Design review of the part built by this model. Coordinates are the model's own, in mm. Face numbers are marked on the shaded views. A direction names the side the tool comes from. Coordinates: 2 decimals unless noted, no trailing zeros. Write each loop counter-clockwise with the first axis right and the second up, starting at its lowest first coordinate (ties: lowest second). Pieces come first, ordered by that corner, then holes.
Q1. For L1, parallel to Y at x = 0, z = 4; L2, parallel to X at y = 14, z = 2.25; L3, parallel to Y at x = -35, z = 6.5, list the stretches that pass through material, from the lowest coordinate up.
Q2. Take a section at A-A, the plane x = 0. Write out the cut boundary in (y, z), plus the area to 3 significant figures.
Q3. For the marked faces 5, 6 and 7, list the 3-axis set-ups (+Z, -Z, +X, -X, +Y, -Y) from which the entire face can be reached by the end or side of a thin tool; tool diameter is ignored.
Q4. Take a section at B-B, the plane z = 4.5. Write out the cut boundary in (x, y), plus the area to 3 significant figures.
Q5. The part is to be moulded in two halves that separate along X. For the marked faces 1, 2, 3 and 4, say which applies: released by +X, released by -X, zero draft, split by the parting line, or undercut.
Q6. For pin 1 Ø5 at (y, z) = (-25.5, 8.5) entering from +X; pin 2 Ø3 at (x, z) = (-21.5, 4.5) entering from +Y; pin 3 Ø3 at (y, z) = (-28.5, 3) entering from -X, all flat-tipped, find the tip position at first contact; note any pin that passes through.
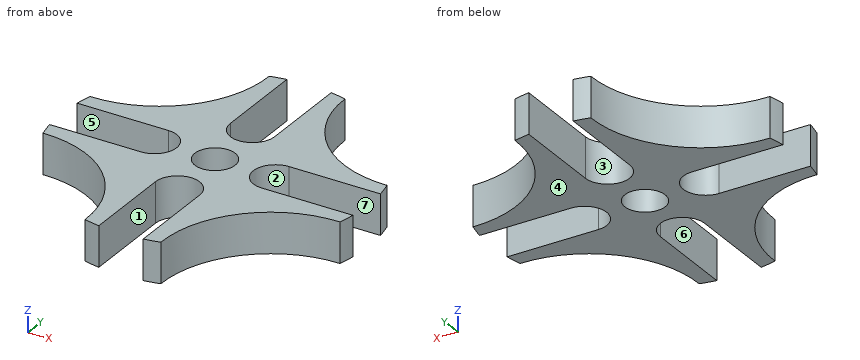
from build123d import *

# Parameters (mm, degrees)
SPIDER_PLATE_PROFILE_R          = 5
SPIDER_PLATE_EXTRUDE_10MM_DEPTH = 10


with BuildPart() as part:
    # Spider Plate Profile → Spider Plate Extrude 10mm (new body)
    with BuildSketch(Plane.XY):
        with BuildLine():
            Line((5.5, -15), (5.5, -37.599867021))
            ThreePointArc((5.5, -37.599867021), (7.46440512, -37.259665272), (9.408264389, -36.816905916))
            ThreePointArc((9.408264389, -36.816905916), (17.313241035, -17.313241035), (36.816905916, -9.408264389))
            ThreePointArc((36.816905916, -9.408264389), (37.259665272, -7.46440512), (37.599867021, -5.5))
            Line((37.599867021, -5.5), (15, -5.5))
            ThreePointArc((15, -5.5), (9.5, 0), (15, 5.5))
            Line((15, 5.5), (37.599867021, 5.5))
            ThreePointArc((37.599867021, 5.5), (37.259665272, 7.46440512), (36.816905916, 9.408264389))
            ThreePointArc((36.816905916, 9.408264389), (17.313241035, 17.313241035), (9.408264389, 36.816905916))
            ThreePointArc((9.408264389, 36.816905916), (7.46440512, 37.259665272), (5.5, 37.599867021))
            Line((5.5, 37.599867021), (5.5, 15))
            ThreePointArc((5.5, 15), (0, 9.5), (-5.5, 15))
            Line((-5.5, 15), (-5.5, 37.599867021))
            ThreePointArc((-5.5, 37.599867021), (-7.46440512, 37.259665272), (-9.408264389, 36.816905916))
            ThreePointArc((-9.408264389, 36.816905916), (-17.313241035, 17.313241035), (-36.816905916, 9.408264389))
            ThreePointArc((-36.816905916, 9.408264389), (-37.259665272, 7.46440512), (-37.599867021, 5.5))
            Line((-37.599867021, 5.5), (-15, 5.5))
            ThreePointArc((-15, 5.5), (-9.5, 0), (-15, -5.5))
            Line((-15, -5.5), (-37.599867021, -5.5))
            ThreePointArc((-37.599867021, -5.5), (-37.259665272, -7.46440512), (-36.816905916, -9.408264389))
            ThreePointArc((-36.816905916, -9.408264389), (-17.313241035, -17.313241035), (-9.408264389, -36.816905916))
            ThreePointArc((-9.408264389, -36.816905916), (-7.46440512, -37.259665272), (-5.5, -37.599867021))
            Line((-5.5, -37.599867021), (-5.5, -15))
            ThreePointArc((-5.5, -15), (0, -9.5), (5.5, -15))
        make_face()
        Circle(SPIDER_PLATE_PROFILE_R, mode=Mode.SUBTRACT)
    extrude(amount=SPIDER_PLATE_EXTRUDE_10MM_DEPTH)


solid = part.part
Responses:
1. L1: y = -9.5 to -5, 5 to 9.5
1. L2: x = -21.34 to -5.41, 5.41 to 21.34
1. L3: y = -9.44 to -5.5, 5.5 to 9.44
2. outline: (-9.5, 0) - (-5, 0) - (-5, 10) - (-9.5, 10) - close; (5, 0) - (9.5, 0) - (9.5, 10) - (5, 10) - close
2. area: 90.0 mm2
3. face 5: +Z, -Z, -X
3. face 6: +Z, -Z, -Y
3. face 7: +Z, -Z, +X
4. outline: (-37.6, -5.5) arc R38 ccw to (-36.82, -9.41) arc R27 cw to (-9.41, -36.82) arc R38 ccw to (-5.5, -37.6) - (-5.5, -15) arc R5.5 cw to (5.5, -15) - (5.5, -37.6) arc R38 ccw to (9.41, -36.82) arc R27 cw to (36.82, -9.41) arc R38 ccw to (37.6, -5.5) - (15, -5.5) arc R5.5 cw to (15, 5.5) - (37.6, 5.5) arc R38 ccw to (36.82, 9.41) arc R27 cw to (9.41, 36.82) arc R38 ccw to (5.5, 37.6) - (5.5, 15) arc R5.5 cw to (-5.5, 15) - (-5.5, 37.6) arc R38 ccw to (-9.41, 36.82) arc R27 cw to (-36.82, 9.41) arc R38 ccw to (-37.6, 5.5) - (-15, 5.5) arc R5.5 cw to (-15, -5.5) - close; hole circle Ø10 at (0, 0)
4. area: 1,830 mm2
5. face 1: undercut
5. face 2: released by +X
5. face 3: undercut
5. face 4: zero draft
6. pin 1: stops at x = 12.97
6. pin 2: stops at y = 14.96
6. pin 3: stops at x = -11.1
